Study the drawing (mm; zero at the part's minimum x, y, z) and answer. Give positions to 0.01 mm unless a question says otherwise; leave off trailing zeros. Order: outer loops, then holes, each group sorted by start corner. A loop starts at its lowest first (then second) coordinate and runs counter-clockwise, first axis right, second up. Notation, with made-up numbers: (78.25, 44.5) - (127.25, 44.5) arc R22 ccw to (127.25, 74.5) - close; hole circle Ø2 at (76, 62.5). An arc over 180 degrees is marked (long way). Use CSV: the item, a comma, the result in double quotes.
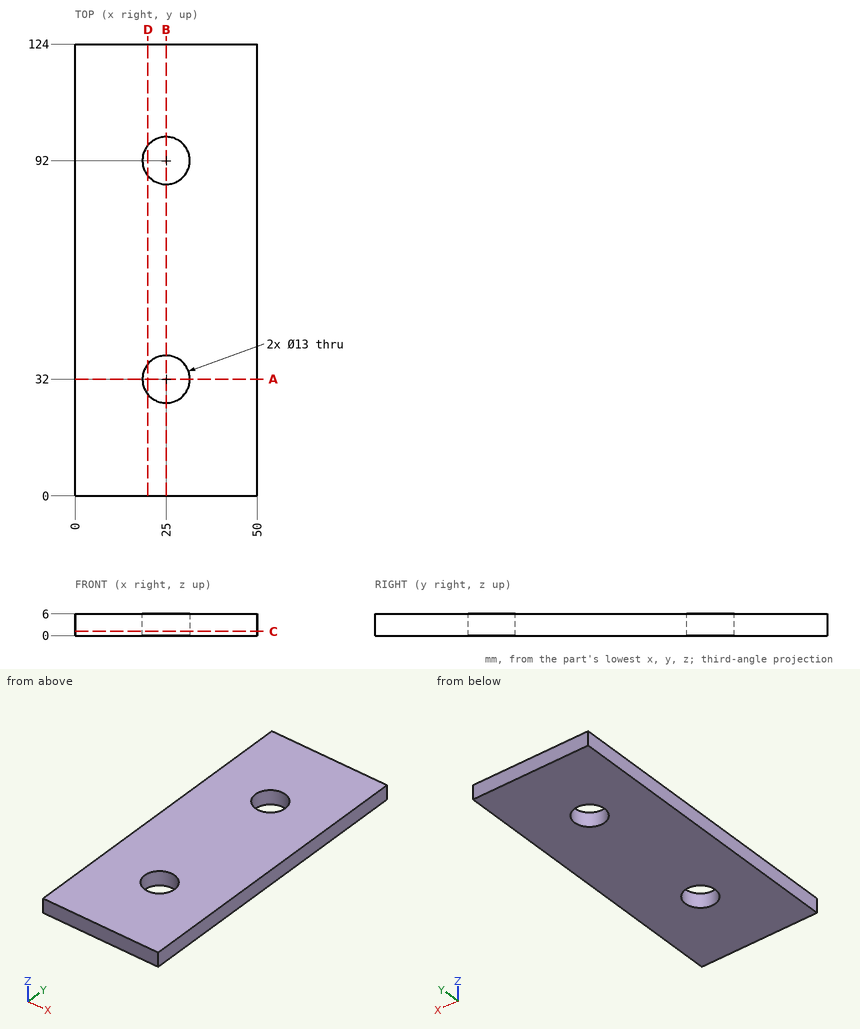
Item 1: The part is cut by section B-B (x = 25). Give the vertices of the cut face in (y, z).
Taken from the geometry:
outline,"(0, 0) - (25.5, 0) - (25.5, 6) - (0, 6) - close; (38.5, 0) - (85.5, 0) - (85.5, 6) - (38.5, 6) - close; (98.5, 0) - (124, 0) - (124, 6) - (98.5, 6) - close"
Item 2: The part is cut by section D-D (x = 20). Give the vertices of the cut face in (y, z).
Taken from the geometry:
outline,"(0, 0) - (27.85, 0) - (27.85, 6) - (0, 6) - close; (36.15, 0) - (87.85, 0) - (87.85, 6) - (36.15, 6) - close; (96.15, 0) - (124, 0) - (124, 6) - (96.15, 6) - close"
Item 3: The part is cut by section A-A (y = 32). Give the vertices of the cut face in (x, z).
Taken from the geometry:
outline,"(0, 0) - (18.5, 0) - (18.5, 6) - (0, 6) - close; (31.5, 0) - (50, 0) - (50, 6) - (31.5, 6) - close"
Item 4: The part is cut by section C-C (z = 1.2). Give the vertices of the cut face in (x, y).
Taken from the geometry:
outline,"(0, 0) - (50, 0) - (50, 124) - (0, 124) - close; hole circle Ø13 at (25, 32); hole circle Ø13 at (25, 92)"
Item 5: Find the intervals of material crossed by line 1 along Y through (x, z) = (25, 3.6); line 2 along Y through (x, z) = (30, 0.7), in increasing order.
Taken from the geometry:
line 1,"0 to 25.5, 38.5 to 85.5, 98.5 to 124"
line 2,"0 to 27.85, 36.15 to 87.85, 96.15 to 124"
